CAD build for the part. Positions are in the model's coordinates, mm. A direction names the side the tool comes from. Round coordinates to 2 decimals unless told otherwise and drop trailing zeros. Order: outer loops, then holes, each group sorted by start corner. A loop starts at its lowest first (then second) coordinate and runs counter-clockwise, first axis right, second up. Notation, with made-up numbers: (49.5, 72) -> (101.5, 72) arc R16 cw to (101.5, 87) -> close; hole circle Ø4 at (27, 44.5). An arc over 180 degrees is marked (long way). Return JSON: item names as keys, results as strings. Group by question number.
Q1. Flat gauge pins, fed straight in: pin 1 (8 mm diameter, centred on y = -4, z = 25, fed in from +X); pin 2 (3 mm diameter, centred on y = -12.5, z = -29, fed in from +X); pin 3 (4.5 mm diameter, centred on y = 35.5, z = -29, fed in from +X). Where does each tip first touch, or does it go through?
Q2. Cut at C-C (z = 25). Write the cut outline in (x, y), then the cut area to 3 significant figures.
Q3. Cut at D-D (y = -35). Write the cut outline in (x, z), then the cut area to 3 significant figures.
Q4. Cut at B-B (y = -4). Write the cut outline in (x, z), then the cut area to 3 significant figures.
Q5. Mould opens along Y. For faces 1 (the flat face through (6.3, -6.2, -27.2)), 2 (the flat face through (6, 60, 0)), 3 (the flat face through (0, 1, 0)) say: +Y half, -Y half, draft (parallel to the pull), parting line (faces both ways), or undercut.
Q6. Which spindle directions (+Z, -Z, +X, -X, +Y, -Y) get a long thin tool onto all of the face, cutting with end or side? Do faces 4 (the cylindrical face through (9, -4, -20)), 5 (the flat face through (6, -1, -35)). Say none if no direction does.
Q7. Cut at A-A (x = 10.25). Count the separate pieces of the cut face and the enclosed holes in it, then the cut area to 3 significant figures.
Q8. Probe line 1 along Z through (x, y) = (5, -12.5); line 2 along Y through (x, z) = (8.1, 25); line 3 along Y through (x, z) = (11.5, 0). List the from-to ranges inside material, lowest first.
from build123d import *

# Parameters (mm, degrees)
SKETCH1_W                                            = 70
SKETCH1_H                                            = 120
BOSS_EXTRUDE1_DEPTH                                  = 12
M5_TAPPED_HOLE1_D                                    = 4.2
M5_TAPPED_HOLE1_DEPTH                                = 12.4
M5_TAPPED_HOLE1_TIP                                  = 1.2618073
CBORE_FOR_M5_HEXAGON_SOCKET_HEAD_CAP_SCR_D           = 5.5
CBORE_FOR_M5_HEXAGON_SOCKET_HEAD_CAP_SCR_CBORE_D     = 10
CBORE_FOR_M5_HEXAGON_SOCKET_HEAD_CAP_SCR_CBORE_DEPTH = 5.7
M4_TAPPED_HOLE1_D                                    = 3.3
M4_TAPPED_HOLE1_DEPTH                                = 10.1
M4_TAPPED_HOLE1_TIP                                  = 0.991420021
F_5_0MM_DOWEL_HOLE1_D                                = 5
F_5_0MM_DOWEL_HOLE1_DEPTH                            = 8
F_5_0MM_DOWEL_HOLE1_TIP                              = 1.502151548
CHAMFER1_SIZE                                        = 2


with BuildPart() as part:
    # Sketch1 → Boss-Extrude1 (new body)
    with BuildSketch(Plane(origin=(0, 0, 0), x_dir=(0, 0, -1), z_dir=(1, 0, 0))):
        Rectangle(SKETCH1_W, SKETCH1_H)
    extrude(amount=BOSS_EXTRUDE1_DEPTH)

    # M5 Tapped Hole1
    with Locations(Plane.ZY):
        with Locations((0, -35), (0, -55)):
            Hole(M5_TAPPED_HOLE1_D / 2, depth=M5_TAPPED_HOLE1_DEPTH)
            with Locations((0, 0, -(M5_TAPPED_HOLE1_DEPTH + M5_TAPPED_HOLE1_TIP / 2))):  # 118° drill point
                Cone(0, M5_TAPPED_HOLE1_D / 2, M5_TAPPED_HOLE1_TIP, mode=Mode.SUBTRACT)

    # CBORE for M5 Hexagon socket head cap screws1 (through all)
    with Locations(Plane(origin=(12, 0, 0), x_dir=(0, 0, -1), z_dir=(1, 0, 0))):
        with Locations((25, -4), (-25, -4)):
            CounterBoreHole(CBORE_FOR_M5_HEXAGON_SOCKET_HEAD_CAP_SCR_D / 2, CBORE_FOR_M5_HEXAGON_SOCKET_HEAD_CAP_SCR_CBORE_D / 2, CBORE_FOR_M5_HEXAGON_SOCKET_HEAD_CAP_SCR_CBORE_DEPTH)

    # M4 Tapped Hole1
    with Locations(Plane(origin=(12, 0, 0), x_dir=(0, 0, -1), z_dir=(1, 0, 0))):
        with Locations((0, -48.5), (0, -12.5), (0, 35.5)):
            Hole(M4_TAPPED_HOLE1_D / 2, depth=M4_TAPPED_HOLE1_DEPTH)
            with Locations((0, 0, -(M4_TAPPED_HOLE1_DEPTH + M4_TAPPED_HOLE1_TIP / 2))):  # 118° drill point
                Cone(0, M4_TAPPED_HOLE1_D / 2, M4_TAPPED_HOLE1_TIP, mode=Mode.SUBTRACT)

    # Ø5.0mm Dowel Hole1
    with Locations(Plane(origin=(12, 0, 0), x_dir=(0, 0, -1), z_dir=(1, 0, 0))):
        with Locations((29, 35.5), (29, -12.5)):
            Hole(F_5_0MM_DOWEL_HOLE1_D / 2, depth=F_5_0MM_DOWEL_HOLE1_DEPTH)
            with Locations((0, 0, -(F_5_0MM_DOWEL_HOLE1_DEPTH + F_5_0MM_DOWEL_HOLE1_TIP / 2))):  # 118° drill point
                Cone(0, F_5_0MM_DOWEL_HOLE1_D / 2, F_5_0MM_DOWEL_HOLE1_TIP, mode=Mode.SUBTRACT)

    # Chamfer1
    chamfer1_edges = [part.edges().sort_by_distance(p)[0] for p in [
        (6, -60, -35),
        (6, -60, 35),
        (6, 60, 35),
        (6, 60, -35),
    ]]
    chamfer(chamfer1_edges, length=CHAMFER1_SIZE)


solid = part.part
Solution:
{
 "1": {"pin 1": "stops at x = 6.3", "pin 2": "stops at x = 3.4", "pin 3": "stops at x = 3.85"},
 "2": {"outline": "(0, -60) -> (12, -60) -> (12, -9) -> (6.3, -9) -> (6.3, -6.75) -> (0, -6.75) -> close; (0, -1.25) -> (6.3, -1.25) -> (6.3, 1) -> (12, 1) -> (12, 60) -> (0, 60) -> close", "area": "1,350 mm²"},
 "3": {"outline": "(0, -35) -> (12, -35) -> (12, -2.1) -> (0, -2.1) -> close; (0, 2.1) -> (12, 2.1) -> (12, 35) -> (0, 35) -> close", "area": "790 mm²"},
 "4": {"outline": "(0, -35) -> (12, -35) -> (12, -30) -> (6.3, -30) -> (6.3, -27.75) -> (0, -27.75) -> close; (0, -22.25) -> (6.3, -22.25) -> (6.3, -20) -> (12, -20) -> (12, 20) -> (6.3, 20) -> (6.3, 22.25) -> (0, 22.25) -> close; (0, 27.75) -> (6.3, 27.75) -> (6.3, 30) -> (12, 30) -> (12, 35) -> (0, 35) -> close", "area": "657 mm²"},
 "5": {"face 1": "undercut", "face 2": "+Y half", "face 3": "draft"},
 "6": {"face 4": "+X", "face 5": "-Z, +X, -X, +Y, -Y"},
 "7": {"separate pieces": "1", "enclosed holes": "9", "area": "8,140 mm²"},
 "8": {"line 1": "z = -35 to -31.5, -26.5 to -1.65, 1.65 to 35", "line 2": "y = -60 to -9, 1 to 60", "line 3": "y = -60 to -57.1, -52.9 to -50.15, -46.85 to -37.1, -32.9 to -14.15, -10.85 to 33.85, 37.15 to 60"}
}
